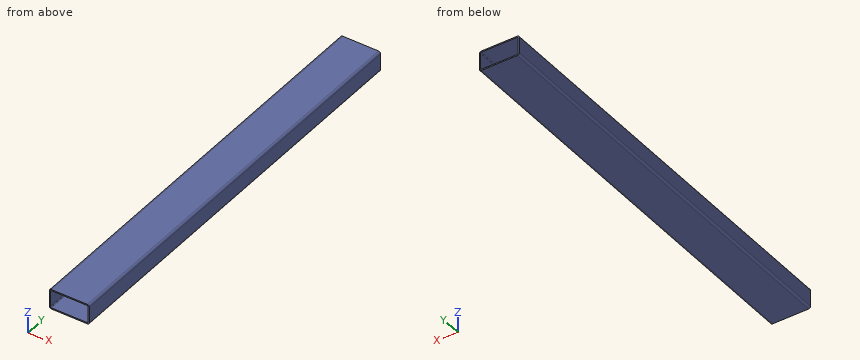
from build123d import *

# Parameters (mm, degrees)
EXTRUDE_THIN1_DEPTH = 1057


with BuildPart() as part:
    # Sketch1 → Extrude-Thin1 (new, symmetric)
    with BuildSketch(Plane(origin=(0, 0, 0), x_dir=(1, 0, 0), z_dir=(0, 1, 0))):
        with BuildLine():
            Line((-90, 50), (90, 50))
            ThreePointArc((90, 50), (97.071067812, 47.071067812), (100, 40))
            Line((100, 40), (100, -40))
            ThreePointArc((100, -40), (97.071067812, -47.071067812), (90, -50))
            Line((90, -50), (-90, -50))
            ThreePointArc((-90, -50), (-97.071067812, -47.071067812), (-100, -40))
            Line((-100, -40), (-100, 40))
            ThreePointArc((-100, 40), (-97.071067812, 47.071067812), (-90, 50))
        make_face()
        with BuildLine():
            Line((-90, 44), (90, 44))
            ThreePointArc((90, 44), (92.828427125, 42.828427125), (94, 40))
            Line((94, 40), (94, -40))
            ThreePointArc((94, -40), (92.828427125, -42.828427125), (90, -44))
            Line((90, -44), (-90, -44))
            ThreePointArc((-90, -44), (-92.828427125, -42.828427125), (-94, -40))
            Line((-94, -40), (-94, 40))
            ThreePointArc((-94, 40), (-92.828427125, 42.828427125), (-90, 44))
        make_face(mode=Mode.SUBTRACT)
    extrude(amount=EXTRUDE_THIN1_DEPTH, both=True)


solid = part.part
The model under review builds one solid part; all positions refer to its coordinate system, in mm. Coordinates: 2 decimals unless noted, no trailing zeros. Loops run counter-clockwise (first coordinate to the right, second up) from the corner with the lowest first, then second, coordinate; pieces in that order, holes last. Notation, with made-up numbers: (82, -11.5) -> (130, -11.5) arc R11 cw to (130, 8.5) -> close; hole circle Ø3 at (11, 47). An arc over 180 degrees is marked (long way). Use a Markdown table: item, result. Add a question column.
1. Add section C-C on y = -837.5. Write out the cut boundary in (x, z).
2. Add section A-A on z = -2. Write out the cut boundary in (x, y).
3. To check wall thickness, follow line 1 (Z direction, x = -52.5, y = -644); line 2 (X direction, y = 357, z = 32.5); line 3 (X direction, y = -545.5, z = 42). State the ranges of each line that lie inside material, in increasing order.
4. Add section B-B on x = -14. Write out the cut boundary in (y, z).
Returned:
| question | item | result |
|---|---|---|
| 1 | outline | (-100, -40) arc R10 ccw to (-90, -50) -> (90, -50) arc R10 ccw to (100, -40) -> (100, 40) arc R10 ccw to (90, 50) -> (-90, 50) arc R10 ccw to (-100, 40) -> close; hole (-94, -40) arc R4 ccw to (-90, -44) -> (90, -44) arc R4 ccw to (94, -40) -> (94, 40) arc R4 ccw to (90, 44) -> (-90, 44) arc R4 ccw to (-94, 40) -> close |
| 2 | outline | (-100, -1057) -> (-94, -1057) -> (-94, 1057) -> (-100, 1057) -> close; (94, -1057) -> (100, -1057) -> (100, 1057) -> (94, 1057) -> close |
| 3 | line 1 | z = -50 to -44, 44 to 50 |
| 3 | line 2 | x = -100 to -94, 94 to 100 |
| 3 | line 3 | x = -99.8 to -93.46, 93.46 to 99.8 |
| 4 | outline | (-1057, -50) -> (1057, -50) -> (1057, -44) -> (-1057, -44) -> close; (-1057, 44) -> (1057, 44) -> (1057, 50) -> (-1057, 50) -> close |
